from build123d import *

# Parameters (mm, degrees)
SKETCH1_W           = 180
SKETCH1_H           = 320
BOSS_EXTRUDE1_DEPTH = 10
SKETCH2_W           = 60
SKETCH2_H           = 130
CUT_EXTRUDE1_DEPTH  = 184.847763109
FILLET1_R           = 8
SKETCH3_W           = 45
SKETCH3_H           = 10
BOSS_EXTRUDE2_DEPTH = 120


with BuildPart() as part:
    # Sketch1 → Boss-Extrude1 (new body)
    with BuildSketch(Plane(origin=(0, 0, 0), x_dir=(1, 0, 0), z_dir=(0, 1, 0))):
        Rectangle(SKETCH1_W, SKETCH1_H)
    extrude(amount=BOSS_EXTRUDE1_DEPTH)

    # Sketch2 → Cut-Extrude1 (cut, through all)
    with BuildSketch(Plane(origin=(0, 10, 0), x_dir=(1, 0, 0), z_dir=(0, 1, 0))):
        with Locations((0, -75)):
            Rectangle(SKETCH2_W, SKETCH2_H)
    extrude(amount=-CUT_EXTRUDE1_DEPTH, mode=Mode.SUBTRACT)

    # Fillet1
    fillet1_edges = [part.edges().sort_by_distance(p)[0] for p in [
        (30, 5, 10),
        (30, 5, 140),
        (-30, 5, 140),
        (-30, 5, 10),
    ]]
    fillet(fillet1_edges, radius=FILLET1_R)

    # Sketch3 → Boss-Extrude2 (add)
    with BuildSketch(Plane(origin=(90, 0, 0), x_dir=(0, 0, -1), z_dir=(1, 0, 0))):
        with Locations((-137.5, 5)):
            Rectangle(SKETCH3_W, SKETCH3_H)
    extrude(amount=BOSS_EXTRUDE2_DEPTH)


solid = part.part
Geometry: final body of the model. Coordinates: model frame, mm. A direction names the side the tool comes from. Give positions to 0.01 mm unless a question says otherwise; leave off trailing zeros. Loops run counter-clockwise (first coordinate to the right, second up) from the corner with the lowest first, then second, coordinate; pieces in that order, holes last. Notation, with made-up numbers: M -13.5,23.5 L 38.5,23.5 A25 cw 38.5,53.5 Z; hole C 60,76.25 d1. An arc over 180 degrees is marked long. Put each result on its own line as item: value.
1) Cut plane B-B, the plane z = 70. Return the cut outline in (x, y).
Computed values:
outline: M -90,0 L -30,0 L -30,10 L -90,10 Z; M 30,0 L 90,0 L 90,10 L 30,10 Z
2) Cut plane A-A, the plane x = -6.5. Return the cut outline in (y, z), plus the area to 3 significant figures.
Computed values:
outline: M 0,-160 L 10,-160 L 10,10 L 0,10 Z; M 0,140 L 10,140 L 10,160 L 0,160 Z
area: 1,900 mm^2
3) Cut plane C-C, the plane y = 1.75. Return the cut outline in (x, z).
Computed values:
outline: M -90,-160 L 90,-160 L 90,115 L 210,115 L 210,160 L -90,160 Z; hole M -30,18 A8 ccw -22,10 L 22,10 A8 ccw 30,18 L 30,132 A8 ccw 22,140 L -22,140 A8 ccw -30,132 Z
4) Cut plane D-D, the plane z = -126. Return the cut outline in (x, y), plus the area to 3 significant figures.
Computed values:
outline: M -90,0 L 90,0 L 90,10 L -90,10 Z
area: 1,800 mm^2
5) Mould query, pull axis X, two halves, no side actions, for faces 1 (the cylindrical face through (-27.594, 4.93, 12.281)), 2 (the flat face through (-1, 5, -160)), 3 (the flat face through (90, 5, -21)). Classes: released by +X, released by -X, zero draft, split by the parting line, or undercut.
Computed values:
face 1: undercut
face 2: zero draft
face 3: released by +X
6) First-contact query: P1, Ø4, axis at y = 5.5, z = 82, coming from the +X side; P2, Ø3, axis at x = 138.5, y = 4.5, coming from the -Z side. Flat tips, straight axial feed; report the tip coordinate or a pass-through.
Computed values:
P1: stops at x = 90
P2: stops at z = 115
7) Material intervals for L1, parallel to Z at x = 21, y = 3.75; L2, parallel to X at y = 7.5, z = 42; L3, parallel to X at y = 5.25, z = -24, sorted ascending. Write a range as from..to.
Computed values:
L1: z = -160..10, 140..160
L2: x = -90..-30, 30..90
L3: x = -90..90
8) Reachability of faces 4 (the flat face through (149, 5, 115)), 5 (the flat face through (30, 5, 76)), 6 (the flat face through (-90, 5, 2)) from +Z, -Z, +X, -X, +Y, -Y: full face, straight path, thin tool, end or side. Return the list, or none.
Computed values:
face 4: -Z, +X, +Y, -Y
face 5: +Y, -Y
face 6: +Z, -Z, -X, +Y, -Y
